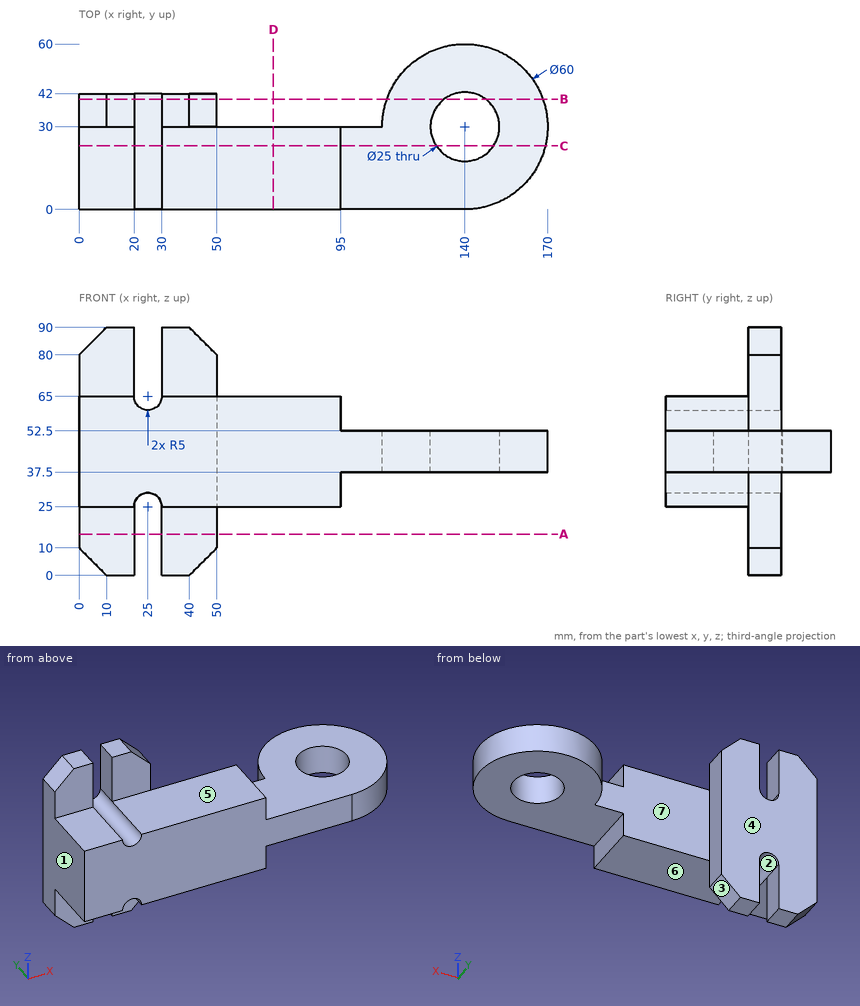
For this review, use the dimensioned drawing (mm, ordinates from the lowest corner) and the shaded views. A direction names the side the tool comes from. Give positions to 0.01 mm unless a question says otherwise; leave off trailing zeros. Write each loop counter-clockwise with the first axis right and the second up, starting at its lowest first coordinate (ties: lowest second). Pieces come first, ordered by that corner, then holes.
(1) Tool access review of the marked faces 5, 6 and 7: name each direction out of +Z, -Z, +X, -X, +Y, -Y from which nothing blocks a thin tool from reaching the whole face with its end or side.
(2) To check wall thickness, follow L1, parallel to Y at x = 140, z = 47.75; L2, parallel to X at y = 32, z = 16.5; L3, parallel to Y at x = 25, z = 55. State the ranges of each line that lie inside material, in increasing order.
(3) Consider section B-B, the plane y = 40. Give the boundary of the cut face in (x, z).
(4) Consider section A-A, the plane z = 15. Give the boundary of the cut face in (x, y), and give its area (3 significant figures).
(5) For P1, Ø2, axis at x = 96, z = 41, coming from the +Y side; P2, Ø4, axis at y = 45, z = 44.5, coming from the +X side; P3, Ø10, axis at x = 149, z = 41, coming from the +Y side; P4, Ø12, axis at x = 94.5, z = 72, coming from the -Y side, all flat-tipped, find the tip position at first contact; note any pin that passes through.
(6) Consider section D-D, the plane x = 70.5. Give the boundary of the cut face in (y, z), and give its area (3 significant figures).
(7) Consider section C-C, the plane y = 23. Give the boundary of the cut face in (x, z), and give its area (3 significant figures).
(8) The part is to be moulded in two halves that separate along X. For the marked faces 1, 2, 3 and 4, say which applies: released by +X, released by -X, zero draft, split by the parting line, or undercut.
Returned:
1. face 5: +Z, +X, -X, -Y
1. face 6: -Z, +X, -X, -Y
1. face 7: +Z, -Z, +Y
2. L1: y = 0 to 17.5, 42.5 to 60
2. L2: x = 0 to 20, 30 to 50
2. L3: y = 0 to 42
3. outline: (0, 10) - (10, 0) - (20, 0) - (20, 25) arc R5 cw to (30, 25) - (30, 0) - (40, 0) - (50, 10) - (50, 80) - (40, 90) - (30, 90) - (30, 65) arc R5 cw to (20, 65) - (20, 90) - (10, 90) - (0, 80) - close; (111.72, 37.5) - (132.5, 37.5) - (132.5, 52.5) - (111.72, 52.5) - close; (147.5, 37.5) - (168.28, 37.5) - (168.28, 52.5) - (147.5, 52.5) - close
4. outline: (0, 30) - (20, 30) - (20, 42) - (0, 42) - close; (30, 30) - (50, 30) - (50, 42) - (30, 42) - close
4. area: 480 mm2
5. P1: stops at y = 30
5. P2: stops at x = 167.04
5. P3: stops at y = 59.73
5. P4: passes through
6. outline: (0, 25) - (30, 25) - (30, 65) - (0, 65) - close
6. area: 1,200 mm2
7. outline: (0, 25) - (20, 25) arc R5 cw to (30, 25) - (95, 25) - (95, 37.5) - (129.64, 37.5) - (129.64, 52.5) - (95, 52.5) - (95, 65) - (30, 65) arc R5 cw to (20, 65) - (0, 65) - close; (150.36, 37.5) - (169.17, 37.5) - (169.17, 52.5) - (150.36, 52.5) - close
7. area: 4,520 mm2
8. face 1: released by -X
8. face 2: undercut
8. face 3: released by +X
8. face 4: zero draft
